Design review of the part built by this model. Coordinates are the model's own, in mm. A direction names the side the tool comes from. Give positions to 0.01 mm unless a question says otherwise; leave off trailing zeros. Loops run counter-clockwise (first coordinate to the right, second up) from the corner with the lowest first, then second, coordinate; pieces in that order, holes last. Notation, with made-up numbers: M 67,-14 L 121,-14 A16 cw 121,-4 Z; hole C 53,87 d8. An arc over 180 degrees is marked long. Use a Markdown table: item, result. Add a question column.
(1) For faces 1 (the face through (0, 0, 0)), 2 (the face through (-5, 5.6, 8)), list the 3-axis set-ups (+Z, -Z, +X, -X, +Y, -Y) from which the entire face can be reached by the end or side of a thin tool; tool diameter is ignored.
(2) Insertion check: pin 1 Ø4 at (x, z) = (7, 4.5) entering from +Y; pin 2 Ø2.5 at (x, z) = (-7.5, 6) entering from +Y. Each pin has a flat end and moves straight along its axis. Give the tip position at first contact, or say it passes through.
(3) Add section C-C, the plane z = 8.75. Give the boundary of the cut face in (x, y).
(4) For probe 1 along Z at (x, y) = (-7, 2); probe 2 along X at (y, z) = (7.75, 3); probe 3 along Z at (x, y) = (-7, 8.15), list the stretches that pass through material, from the lowest coordinate up.
(5) Add section B-B, the plane y = 6.5. Give the boundary of the cut face in (x, z).
(6) Add section A-A, the plane x = -7. Give the boundary of the cut face in (y, z).
(7) Add section D-D, the plane y = -7.25. Give the boundary of the cut face in (x, z), then the cut area to 3 significant figures.
(8) Draft analysis for pull direction X (two halves, no side actions). For faces 3 (the face through (-9.146, -2.309, 5.324)), 4 (the face through (-12, -0.1, 0.5)), 5 (the face through (6.133, 7.831, 9.905)), 6 (the face through (12.5, 0, 6)), state which applies: pulls with the +X half, pulls with the -X half, needs draft (parallel to the pull), parting line crosses it, or undercut.
```python
from build123d import *

# Parameters (mm, degrees)
SKETCH1_W                                           = 25
SKETCH1_H                                           = 20
BOSS_EXTRUDE1_DEPTH                                 = 12
CBORE_FOR_M4_HEX_SOCKET_HEAD_CAP_SCREW1_D           = 4.5
CBORE_FOR_M4_HEX_SOCKET_HEAD_CAP_SCREW1_CBORE_D     = 8
CBORE_FOR_M4_HEX_SOCKET_HEAD_CAP_SCREW1_CBORE_DEPTH = 4.4
CHAMFER1_SIZE                                       = 1


with BuildPart() as part:
    # Sketch1 → Boss-Extrude1 (new body)
    with BuildSketch(Plane.XY):
        Rectangle(SKETCH1_W, SKETCH1_H)
    extrude(amount=BOSS_EXTRUDE1_DEPTH)

    # CBORE for M4 Hex Socket Head Cap Screw1 (through all)
    with Locations(Plane(origin=(0, 10, 0), x_dir=(1, 0, 0), z_dir=(0, 1, 0))):
        with Locations((-7, -6), (7, -6)):
            CounterBoreHole(CBORE_FOR_M4_HEX_SOCKET_HEAD_CAP_SCREW1_D / 2, CBORE_FOR_M4_HEX_SOCKET_HEAD_CAP_SCREW1_CBORE_D / 2, CBORE_FOR_M4_HEX_SOCKET_HEAD_CAP_SCREW1_CBORE_DEPTH)

    # Chamfer1
    chamfer1_edges = [part.edges().sort_by_distance(p)[0] for p in [
        (-12.5, 0, 12),
        (12.5, 0, 12),
        (-12.5, 0, 0),
        (12.5, 0, 0),
    ]]
    chamfer(chamfer1_edges, length=CHAMFER1_SIZE)


solid = part.part
```
Established:
| question | item | result |
|---|---|---|
| 1 | face 1 | -Z, +X, -X, +Y, -Y |
| 1 | face 2 | +Y |
| 2 | pin 1 | y = 5.6 |
| 2 | pin 2 | through |
| 3 | outline | M -12.5,-10 L 12.5,-10 L 12.5,10 L 9.9,10 L 9.9,5.6 L 4.1,5.6 L 4.1,10 L -4.1,10 L -4.1,5.6 L -9.9,5.6 L -9.9,10 L -12.5,10 Z |
| 4 | probe 1 | 0 to 3.75, 8.25 to 12 |
| 4 | probe 2 | -12.5 to -9.65, -4.35 to 4.35, 9.65 to 12.5 |
| 4 | probe 3 | 0 to 2, 10 to 12 |
| 5 | outline | M -12.5,1 L -11.5,0 L 11.5,0 L 12.5,1 L 12.5,11 L 11.5,12 L -11.5,12 L -12.5,11 Z; hole C -7,6 d8; hole C 7,6 d8 |
| 6 | outline | M -10,0 L 10,0 L 10,2 L 5.6,2 L 5.6,3.75 L -10,3.75 Z; M -10,8.25 L 5.6,8.25 L 5.6,10 L 10,10 L 10,12 L -10,12 Z |
| 7 | outline | M -12.5,1 L -11.5,0 L 11.5,0 L 12.5,1 L 12.5,11 L 11.5,12 L -11.5,12 L -12.5,11 Z; hole C -7,6 d4.5; hole C 7,6 d4.5 |
| 7 | area | 266 mm^2 |
| 8 | face 3 | undercut |
| 8 | face 4 | pulls with the -X half |
| 8 | face 5 | undercut |
| 8 | face 6 | pulls with the +X half |
